Part model, mm, in its own coordinate system. Face numbers are marked on the shaded views. A direction names the side the tool comes from. Round coordinates to 2 decimals unless told otherwise and drop trailing zeros. Use one line per item in the form item = value. Start each with the question number.
Item 1: Probe L1, parallel to X at y = -87.5, z = 4.75; L2, parallel to Y at x = 0.5, z = 5; L3, parallel to Y at x = 0, z = 8. List the from-to ranges inside material, lowest first.
Item 2: Flat gauge pins, fed straight in: pin 1 Ø4.5 at (x, y) = (-20, -67.5) entering from +Z; pin 2 Ø2.5 at (x, y) = (20, -87.5) entering from -Z; pin 3 Ø2.5 at (x, y) = (-1.5, -76.5) entering from +Z. Where does each tip first touch, or does it go through?
Item 3: Which spindle directions (+Z, -Z, +X, -X, +Y, -Y) get a long thin tool onto all of the face, cutting with end or side? Do the marked faces 1 and 2. Say none if no direction does.
from build123d import *

# Parameters (mm, degrees)
SKETCH_1_W                = 80
SKETCH_1_H                = 285
EXTRUDE_1_DEPTH           = 12
HOLE_WIZARD_1_D           = 5.5
HOLE_WIZARD_1_CBORE_D     = 10
HOLE_WIZARD_1_CBORE_DEPTH = 5.7
HOLE_WIZARD_M5_1_D        = 4.2
CUT_EXTRUDE_2_DEPTH       = 2
HOLE_WIZARD_M4_1_D        = 3.3
HOLE_WIZARD_M5_2_D        = 4.2
CHAMFER_2_SIZE            = 2
HOLE_WIZARD_2_D           = 4.5
HOLE_WIZARD_2_CBORE_D     = 8
HOLE_WIZARD_2_CBORE_DEPTH = 6.6


with BuildPart() as part:
    # 草图1 → 凸台-拉伸1 (new body)
    with BuildSketch(Plane.XY):
        Rectangle(SKETCH_1_W, SKETCH_1_H)
    extrude(amount=EXTRUDE_1_DEPTH)

    # 打孔尺寸(%根据)内六角圆柱头螺钉的类型1 (through all)
    with Locations(Plane.XY.offset(12)):
        with Locations((30, 42.5), (-30, 42.5)):
            CounterBoreHole(HOLE_WIZARD_1_D / 2, HOLE_WIZARD_1_CBORE_D / 2, HOLE_WIZARD_1_CBORE_DEPTH)

    # M5 螺纹孔1 (through all)
    with Locations(Plane(origin=(0, 0, 0), x_dir=(-1, 0, 0), z_dir=(0, 0, -1))):
        with Locations((-20, 127.5), (20, 127.5)):
            Hole(HOLE_WIZARD_M5_1_D / 2)

    # 草图25 → 切除-拉伸2 (cut)
    with BuildSketch(Plane.XY.offset(12)):
        with BuildLine():
            Line((-23, -17.5), (23, -17.5))
            ThreePointArc((23, -17.5), (24.414213562, -18.085786438), (25, -19.5))
            Line((25, -19.5), (25, -115.5))
            ThreePointArc((25, -115.5), (24.414213562, -116.914213562), (23, -117.5))
            Line((23, -117.5), (-23, -117.5))
            ThreePointArc((-23, -117.5), (-24.414213562, -116.914213562), (-25, -115.5))
            Line((-25, -115.5), (-25, -19.5))
            ThreePointArc((-25, -19.5), (-24.414213562, -18.085786438), (-23, -17.5))
        make_face()
    extrude(amount=-CUT_EXTRUDE_2_DEPTH, mode=Mode.SUBTRACT)

    # M4 螺纹孔1 (through all)
    with Locations(Plane.XY.offset(10)):
        with Locations((-20, -27.5), (20, -27.5), (20, -37.5), (20, -47.5), (-20, -37.5), (-20, -47.5), (-20, -57.5), (20, -57.5), (-20, -67.5), (20, -67.5), (-20, -77.5), (20, -77.5), (-20, -87.5), (20, -87.5), (-20, -97.5), (20, -97.5), (-20, -107.5), (20, -107.5)):
            Hole(HOLE_WIZARD_M4_1_D / 2)

    # M5 螺纹孔2 (through all)
    with Locations(Plane.XY.offset(12)):
        with Locations((-30, -127.5), (30, -127.5)):
            Hole(HOLE_WIZARD_M5_2_D / 2)

    # 倒角2
    chamfer_2_edges = [part.edges().sort_by_distance(p)[0] for p in [
        (40, -142.5, 6),
        (-40, -142.5, 6),
        (-40, 142.5, 6),
        (40, 142.5, 6),
    ]]
    chamfer(chamfer_2_edges, length=CHAMFER_2_SIZE)

    # 打孔尺寸(%根据)内六角圆柱头螺钉的类型2 (through all)
    with Locations(Plane.XY.offset(12)):
        with Locations((0, 5), (0, -75)):
            CounterBoreHole(HOLE_WIZARD_2_D / 2, HOLE_WIZARD_2_CBORE_D / 2, HOLE_WIZARD_2_CBORE_DEPTH)


solid = part.part
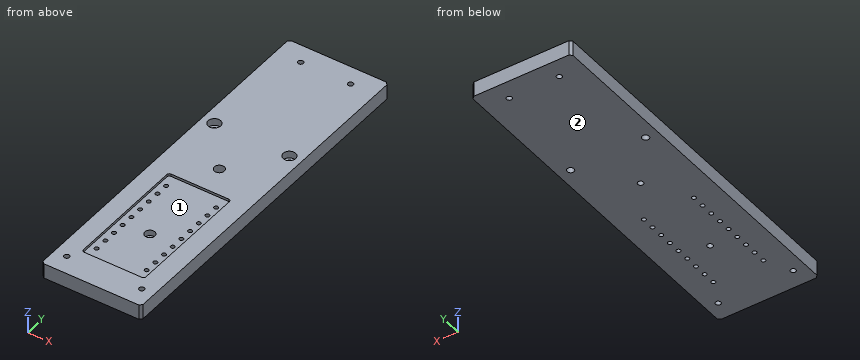
Model answer:
q1.L1 = -40 to -21.65, -18.35 to 18.35, 21.65 to 40
q1.L2 = -142.5 to -77.19, -72.81 to 2.81, 7.19 to 142.5
q1.L3 = -142.5 to -79, -71 to 1, 9 to 142.5
q2.pin_1 = 10
q2.pin_2 = through
q2.pin_3 = 5.4
q3.face_1 = +Z
q3.face_2 = -Z, +X, -X, +Y, -Y
